Geometry: see drawing. Coordinates: mm, zero at the bounding-box minimum. A direction names the side the tool comes from. Round coordinates to 2 decimals unless told otherwise and drop trailing zeros. Write each loop counter-clockwise with the first axis right and the second up, starting at its lowest first coordinate (ties: lowest second). Pieces come first, ordered by that corner, then holes. Notation, with made-up numbers: M 31,25.25 L 73,25.25 A32 cw 73,58.25 Z; hole C 63,-18.75 d11. An arc over 180 degrees is marked long. Use a Markdown table: item, result.
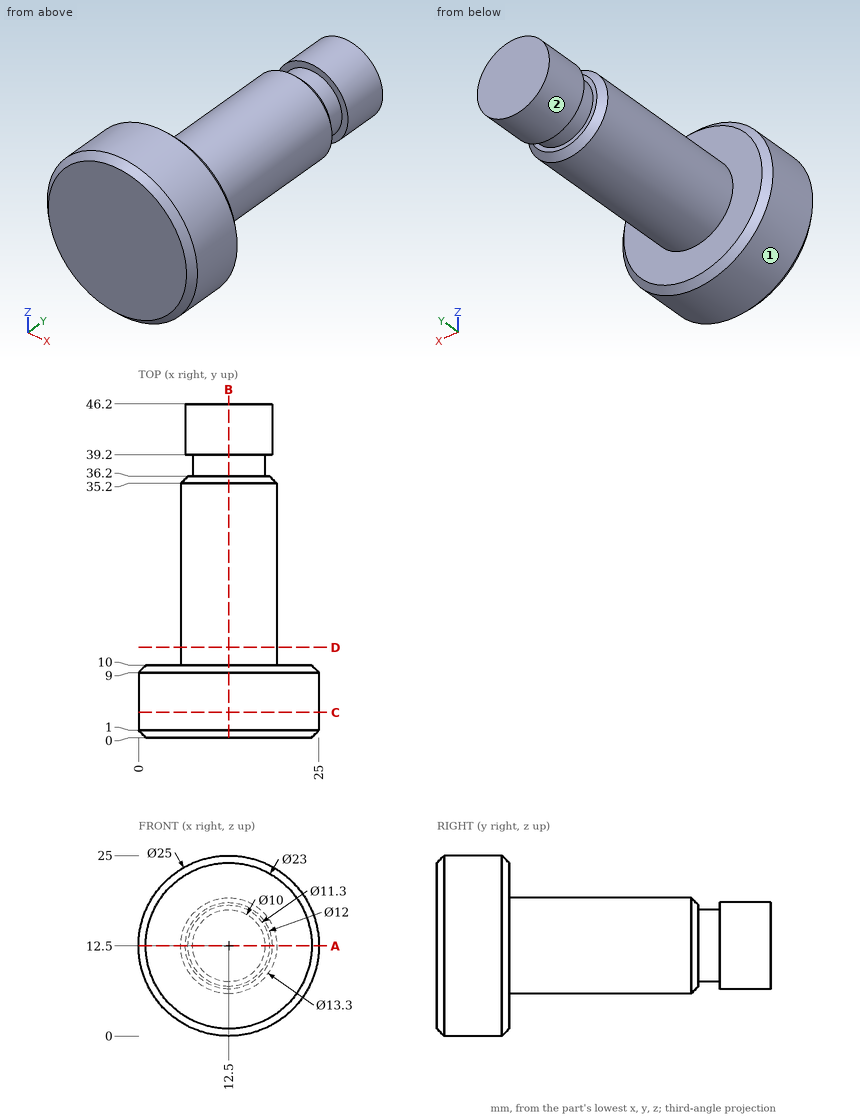
Q1. Section C-C on y = 3.5. Return loops of the section in (x, z), plus the area to 3 significant figures.
Results are:
| item | result |
|---|---|
| outline | C 12.5,12.5 d25 |
| area | 491 mm^2 |
Q2. Section B-B on x = 12.5. Return loops of the section in (y, z), plus the area to 3 significant figures.
Results are:
| item | result |
|---|---|
| outline | M 0,1 L 1,0 L 9,0 L 10,1 L 10,5.85 L 35.2,5.85 L 36.2,6.85 L 36.2,7.5 L 39.2,7.5 L 39.2,6.5 L 46.2,6.5 L 46.2,18.5 L 39.2,18.5 L 39.2,17.5 L 36.2,17.5 L 36.2,18.15 L 35.2,19.15 L 10,19.15 L 10,24 L 9,25 L 1,25 L 0,24 Z |
| area | 709 mm^2 |
Q3. First-contact query: pin 1 Ø3 at (y, z) = (36, 18.5) entering from -X; pin 2 Ø10 at (x, y) = (22, 26.5) entering from -Z; pin 3 Ø5 at (x, y) = (6, 34.5) entering from +Z; pin 4 Ø1.5 at (y, z) = (13.5, 20.5) entering from -X. Flat tips, straight axial feed; report the tip coordinate or a pass-through.
Results are:
| item | result |
|---|---|
| pin 1 | x = 7.83 |
| pin 2 | z = 7.6 |
| pin 3 | z = 17.81 |
| pin 4 | through |
Q4. Line query: L1, parallel to Y at x = 1.5, z = 12.75; L2, parallel to Z at x = 16, y = 20; L3, parallel to Z at x = 12.25, y = 17. Output: solid intervals per line, ascending.
Results are:
| item | result |
|---|---|
| L1 | 0 to 10 |
| L2 | 6.85 to 18.15 |
| L3 | 5.85 to 19.15 |
Q5. Section A-A on z = 12.5. Return loops of the section in (x, y), plus the area to 3 significant figures.
Results are:
| item | result |
|---|---|
| outline | M 0,1 L 1,0 L 24,0 L 25,1 L 25,9 L 24,10 L 19.15,10 L 19.15,35.2 L 18.15,36.2 L 17.5,36.2 L 17.5,39.2 L 18.5,39.2 L 18.5,46.2 L 6.5,46.2 L 6.5,39.2 L 7.5,39.2 L 7.5,36.2 L 6.85,36.2 L 5.85,35.2 L 5.85,10 L 1,10 L 0,9 Z |
| area | 709 mm^2 |
Q6. Reachability of the marked faces 1 and 2 from +Z, -Z, +X, -X, +Y, -Y: full face, straight path, thin tool, end or side. Return the list, or none.
Results are:
| item | result |
|---|---|
| face 1 | +Y, -Y |
| face 2 | +Y |
Q7. Section D-D on y = 12.5. Return loops of the section in (x, z), plus the area to 3 significant figures.
Results are:
| item | result |
|---|---|
| outline | C 12.5,12.5 d13.3 |
| area | 139 mm^2 |
